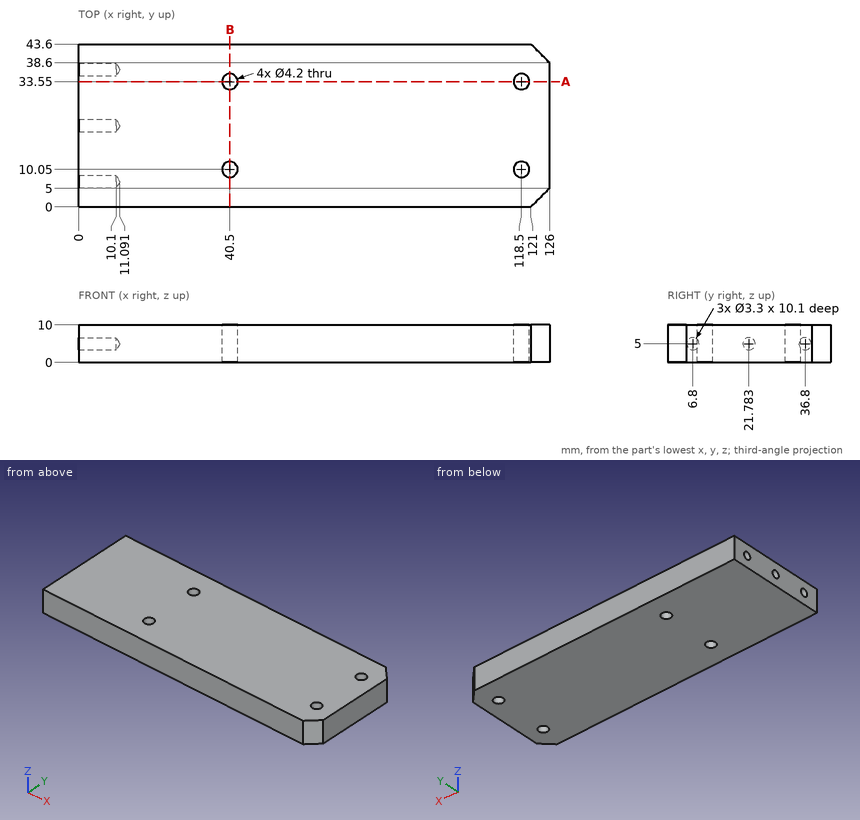
Study the drawing (mm; zero at the part's minimum x, y, z) and answer. Coordinates: 2 decimals unless noted, no trailing zeros. Order: outer loops, then holes, each group sorted by start corner. A loop starts at its lowest first (then second) coordinate and runs counter-clockwise, first axis right, second up. Notation, with made-up numbers: (51.5, 34) -> (106.5, 34) arc R14 cw to (106.5, 43) -> close; hole circle Ø7 at (-32, 29). An arc over 180 degrees is marked (long way). Answer in a Markdown table with one row per item. Add a question column.
Item 1: Each of these flat-tipped pins is pushed along its axis until it touches: P1, Ø2, axis at y = 6.8, z = 5, coming from the -X side; P2, Ø4, axis at x = 40.5, y = 33.55, coming from the +Z side. Where does it stop, or does it pass through?
Item 2: Find section A-A (y = 33.55). Write down the section's boundary in (x, z), then the cut area to 3 significant figures.
Item 3: Find section B-B (x = 40.5). Write down the section's boundary in (y, z), then the cut area to 3 significant figures.
Item 4: Find the intervals of material crossed by L1, parallel to Y at x = 5, z = 5; L2, parallel to Z at x = 5.5, y = 6.8; L3, parallel to Z at x = 10, y = 23 (1 decimal), in increasing order. Write a range as from..to.
Result set:
| question | item | result |
|---|---|---|
| 1 | P1 | stops at x = 10.49 |
| 1 | P2 | passes through |
| 2 | outline | (0, 0) -> (38.4, 0) -> (38.4, 10) -> (0, 10) -> close; (42.6, 0) -> (116.4, 0) -> (116.4, 10) -> (42.6, 10) -> close; (120.6, 0) -> (126, 0) -> (126, 10) -> (120.6, 10) -> close |
| 2 | area | 1,180 mm² |
| 3 | outline | (0, 0) -> (7.95, 0) -> (7.95, 10) -> (0, 10) -> close; (12.15, 0) -> (31.45, 0) -> (31.45, 10) -> (12.15, 10) -> close; (35.65, 0) -> (43.6, 0) -> (43.6, 10) -> (35.65, 10) -> close |
| 3 | area | 352 mm² |
| 4 | L1 | y = 0..5.15, 8.45..20.13, 23.43..35.15, 38.45..43.6 |
| 4 | L2 | z = 0..3.35, 6.65..10 |
| 4 | L3 | z = 0..3.9, 6.1..10 |
